from build123d import *

# Parameters (mm, degrees)
SKETCH1_W           = 80
SKETCH1_H           = 80
BOSS_EXTRUDE1_DEPTH = 38
SKETCH2_W           = 76
SKETCH2_H           = 76
CUT_EXTRUDE1_DEPTH  = 36
SKETCH3_R           = 12.5
CUT_EXTRUDE2_DEPTH  = 10
BOSS_EXTRUDE3_START = 40
SKETCH4_R           = 13.5
SKETCH4_R_2         = 12.5
BOSS_EXTRUDE3_DEPTH = 40


with BuildPart() as part:
    # Sketch1 → Boss-Extrude1 (new body)
    with BuildSketch(Plane(origin=(0, 0, 0), x_dir=(1, 0, 0), z_dir=(0, 1, 0))):
        Rectangle(SKETCH1_W, SKETCH1_H)
    extrude(amount=BOSS_EXTRUDE1_DEPTH)

    # Sketch2 → Cut-Extrude1 (cut)
    with BuildSketch(Plane(origin=(0, 38, 0), x_dir=(1, 0, 0), z_dir=(0, 1, 0))):
        Rectangle(SKETCH2_W, SKETCH2_H)
    extrude(amount=-CUT_EXTRUDE1_DEPTH, mode=Mode.SUBTRACT)

    # Sketch3 → Cut-Extrude2 (cut)
    with BuildSketch(Plane.ZY.offset(40)):
        with Locations((-20, 20)):
            Circle(SKETCH3_R)
        with Locations((20, 20)):
            Circle(SKETCH3_R)
    extrude(amount=-CUT_EXTRUDE2_DEPTH, mode=Mode.SUBTRACT)

    # Sketch4 → Boss-Extrude3 (add)
    # profile 1 of 2: a face of its own
    with BuildSketch(Plane.ZY.offset(40).offset(BOSS_EXTRUDE3_START)):
        with Locations(Location((-20, 20, 0), (0, 0, 180))):
            Circle(SKETCH4_R)
        with Locations((-20, 20)):
            Circle(SKETCH4_R_2, mode=Mode.SUBTRACT)
    # profile 2 of 2: a face of its own
    with BuildSketch(Plane.ZY.offset(40).offset(BOSS_EXTRUDE3_START)):
        with Locations(Location((20, 20, 0), (0, 0, 180))):
            Circle(SKETCH4_R)
        with Locations((20, 20)):
            Circle(SKETCH4_R_2, mode=Mode.SUBTRACT)
    extrude(amount=-BOSS_EXTRUDE3_DEPTH)


solid = part.part
Here's how the part is built. I have some questions about the finished solid (model axes, mm). A direction names the side the tool comes from. Coordinates: 2 decimals unless noted, no trailing zeros. Write each loop counter-clockwise with the first axis right and the second up, starting at its lowest first coordinate (ties: lowest second). Pieces come first, ordered by that corner, then holes.
1) Which directions (+Z, -Z, +X, -X, +Y, -Y) give clear straight access to the entire face, cutting with the end or side of a thin tool? Please do faces 5 (the face through (-38, 20, 1)), 6 (the face through (-59.294, 12.394, -29.92)), 7 (the face through (-3.1, 38, 38.3)).
Filled in:
face 5: +Y
face 6: -X
face 7: +Z, -Z, +X, -X, +Y
2) If we section it at D-D (z = 3): List the corners of the cut face in (x, y) for me.
Filled in:
outline: (-40, 0) - (40, 0) - (40, 38) - (38, 38) - (38, 2) - (-38, 2) - (-38, 38) - (-40, 38) - close
3) If I drill on line 1 (Z direction, x = 26.5, y = 34.5); line 2 (Y direction, x = -63, z = 20), over which ranges is the centre line in solid material (lowest first)?
Filled in:
line 1: z = -40 to -38, 38 to 40
line 2: y = 6.5 to 7.5, 32.5 to 33.5
4) If we section it at C-C (x = -67): List the corners of the cut face in (y, z) for me.
Filled in:
outline: circle Ø27 at (20, -20); circle Ø27 at (20, 20); hole circle Ø25 at (20, -20); hole circle Ø25 at (20, 20)
5) If we section it at B-B (z = -23.5): List the corners of the cut face in (x, y) for me.
Filled in:
outline: (-80, 6.96) - (-40, 6.96) - (-40, 0) - (40, 0) - (40, 38) - (38, 38) - (38, 2) - (-38, 2) - (-38, 8) - (-80, 8) - close; (-80, 32) - (-38, 32) - (-38, 38) - (-40, 38) - (-40, 33.04) - (-80, 33.04) - close
6) If we section it at A-A (y = 20): List the corners of the cut face in (x, z) for me, plus the area to 3 significant figures.
Filled in:
outline: (-80, -33.5) - (-40, -33.5) - (-40, -40) - (40, -40) - (40, 40) - (-40, 40) - (-40, 33.5) - (-80, 33.5) - (-80, 32.5) - (-38, 32.5) - (-38, 38) - (38, 38) - (38, -38) - (-38, -38) - (-38, -32.5) - (-80, -32.5) - close; (-80, -7.5) - (-38, -7.5) - (-38, 7.5) - (-80, 7.5) - (-80, 6.5) - (-40, 6.5) - (-40, -6.5) - (-80, -6.5) - close
area: 684 mm2
7) Thinking about a two-plate mould opening in Z: for faces 1 (the face through (-1, 19, -40)), 2 (the face through (-1, 0, -1)), 3 (the face through (38, 20, 1)), 4 (the face through (-1, 20, -38)), which applies, +Z half, -Z half, draft (parallel to the pull), parting line (faces both ways), or undercut?
Filled in:
face 1: -Z half
face 2: draft
face 3: undercut
face 4: undercut
8) I'm going to push flat-ended pins straight in: pin 1 (12 mm diameter, centred on y = 19, z = 14.5, fed in from -X); pin 2 (23 mm diameter, centred on x = -6, z = -4, fed in from +Y). Where does each tip first touch, or does it pass through?
Filled in:
pin 1: stops at x = 38
pin 2: stops at y = 2
